Geometry: final body of the model. Coordinates: model frame, mm. A direction names the side the tool comes from. Round coordinates to 2 decimals unless told otherwise and drop trailing zeros. Write each loop counter-clockwise with the first axis right and the second up, starting at its lowest first coordinate (ties: lowest second). Pieces come first, ordered by that corner, then holes. Notation, with made-up numbers: M 50.25,71 L 59.25,71 A20 cw 59.25,83 Z; hole C -15,24.5 d5. An arc over 180 degrees is marked long. Put each result on its own line as item: value. Start each with the question number.
```python
from build123d import *

# Parameters (mm, degrees)
F_100_X_100_X_5_1_DEPTH = 200
CUT_EXTRUDE_1_REACH     = 231.129


with BuildPart() as part:
    # Sketch1 → 方形管 100 X 100 X 5   (1) (new body)
    with BuildSketch(Plane(origin=(0, 0, 0), x_dir=(0, 0, -1), z_dir=(1, 0, 0))):
        with BuildLine():
            Line((-40, -50), (40, -50))
            ThreePointArc((40, -50), (47.071067812, -47.071067812), (50, -40))
            Line((50, -40), (50, 40))
            ThreePointArc((50, 40), (47.071067812, 47.071067812), (40, 50))
            Line((40, 50), (-40, 50))
            ThreePointArc((-40, 50), (-47.071067812, 47.071067812), (-50, 40))
            Line((-50, 40), (-50, -40))
            ThreePointArc((-50, -40), (-47.071067812, -47.071067812), (-40, -50))
        make_face()
        with BuildLine():
            Line((-40, -45), (40, -45))
            ThreePointArc((40, -45), (43.535533906, -43.535533906), (45, -40))
            Line((45, -40), (45, 40))
            ThreePointArc((45, 40), (43.535533906, 43.535533906), (40, 45))
            Line((40, 45), (-40, 45))
            ThreePointArc((-40, 45), (-43.535533906, 43.535533906), (-45, 40))
            Line((-45, 40), (-45, -40))
            ThreePointArc((-45, -40), (-43.535533906, -43.535533906), (-40, -45))
        make_face(mode=Mode.SUBTRACT)
    extrude(amount=F_100_X_100_X_5_1_DEPTH)

    # 切除-拉伸1: up to this face of the body (flat: up to its plane)
    cut_extrude_1_end = Plane(part.part.faces().sort_by_distance((100, -50, 0))[0])
    # 草图2 → 切除-拉伸1 (cut, up to the picked face)
    with BuildSketch(Plane.XZ.offset(-50), mode=Mode.PRIVATE) as cut_extrude_1_sk1:
        Polygon((170, 50), (70, -50), (0, -50), (0, 50), align=None)
    cut_extrude_1_tool1 = split(extrude(cut_extrude_1_sk1.sketch, amount=CUT_EXTRUDE_1_REACH, mode=Mode.PRIVATE), bisect_by=cut_extrude_1_end, keep=Keep.BOTH, mode=Mode.PRIVATE)
    add(cut_extrude_1_tool1.solids().sort_by(Axis((63.472222, 50, 6.944444), (0, -1, 0)))[0], mode=Mode.SUBTRACT)


solid = part.part
```
1) Section D-D, the plane x = 126. Output: boundary loops of the cut face in (y, z).
2) Draft query along Z for faces 3 (the face through (200, -48, 4)), 4 (the face through (185, 1, 50)), 5 (the face through (152, 45, -9)), 6 (the face through (152, -45, -8)). Return one class per face: +Z half, -Z half, draft (parallel to the pull), parting line (faces both ways), or undercut.
3) First-contact query: pin 1 (8 mm diameter, centred on x = 89, y = -30, fed in from +Z); pin 2 (12 mm diameter, centred on y = -32.5, z = -36.5, fed in from -X). Flat tips, straight axial feed; report the tip coordinate or a pass-through.
4) Section B-B, the plane x = 177.5. Output: boundary loops of the cut face in (y, z).
5) Ray query, probe 1 along Z at (x, y) = (186, 36); probe 2 along Z at (x, y) = (101.5, -21). Return the intervals inside material, ascending.
6) Section A-A, the plane z = -24. Output: boundary loops of the cut face in (x, y).
7) Access query for faces 1 (the face through (152, -50, -8)), 2 (the face through (180, -43, 44)). Directions: +Z, -Z, +X, -X, +Y, -Y. A direction counts if a zero-diameter tool reaches every point of the face in a straight line with its end or side. Return the directions, or none.
8) Section C-C, the plane y = -38. Output: boundary loops of the cut face in (x, z).
Solved:
1. outline: M -50,-40 A10 ccw -40,-50 L 40,-50 A10 ccw 50,-40 L 50,6 L 45,6 L 45,-40 A5 cw 40,-45 L -40,-45 A5 cw -45,-40 L -45,6 L -50,6 Z
2. face 3: draft
2. face 4: +Z half
2. face 5: undercut
2. face 6: undercut
3. pin 1: stops at z = -45
3. pin 2: passes through
4. outline: M -50,-40 A10 ccw -40,-50 L 40,-50 A10 ccw 50,-40 L 50,40 A10 ccw 40,50 L -40,50 A10 ccw -50,40 Z; hole M -45,-40 A5 ccw -40,-45 L 40,-45 A5 ccw 45,-40 L 45,40 A5 ccw 40,45 L -40,45 A5 ccw -45,40 Z
5. probe 1: z = -50 to -45, 45 to 50
5. probe 2: z = -50 to -45
6. outline: M 96,-50 L 200,-50 L 200,-45 L 96,-45 Z; M 96,45 L 200,45 L 200,50 L 96,50 Z
7. face 1: +Z, -Z, +X, -X, -Y
7. face 2: +X, -X
8. outline: M 70,-50 L 200,-50 L 200,-45 L 75,-45 Z; M 165,45 L 200,45 L 200,50 L 170,50 Z
